Check sheet for the drawn part. Datum: minimum x, y, z corner. Units: mm. Round coordinates to 2 decimals unless told otherwise and drop trailing zeros. Loops run counter-clockwise (first coordinate to the right, second up) from the corner with the lowest first, then second, coordinate; pieces in that order, holes last. Notation, with made-up numbers: (74.5, 70.5) -> (127.5, 70.5) arc R24 cw to (127.5, 85.5) -> close; hole circle Ø5 at (-7, 45). An arc over 180 degrees is marked (long way). Return JSON: item names as keys, results as strings.
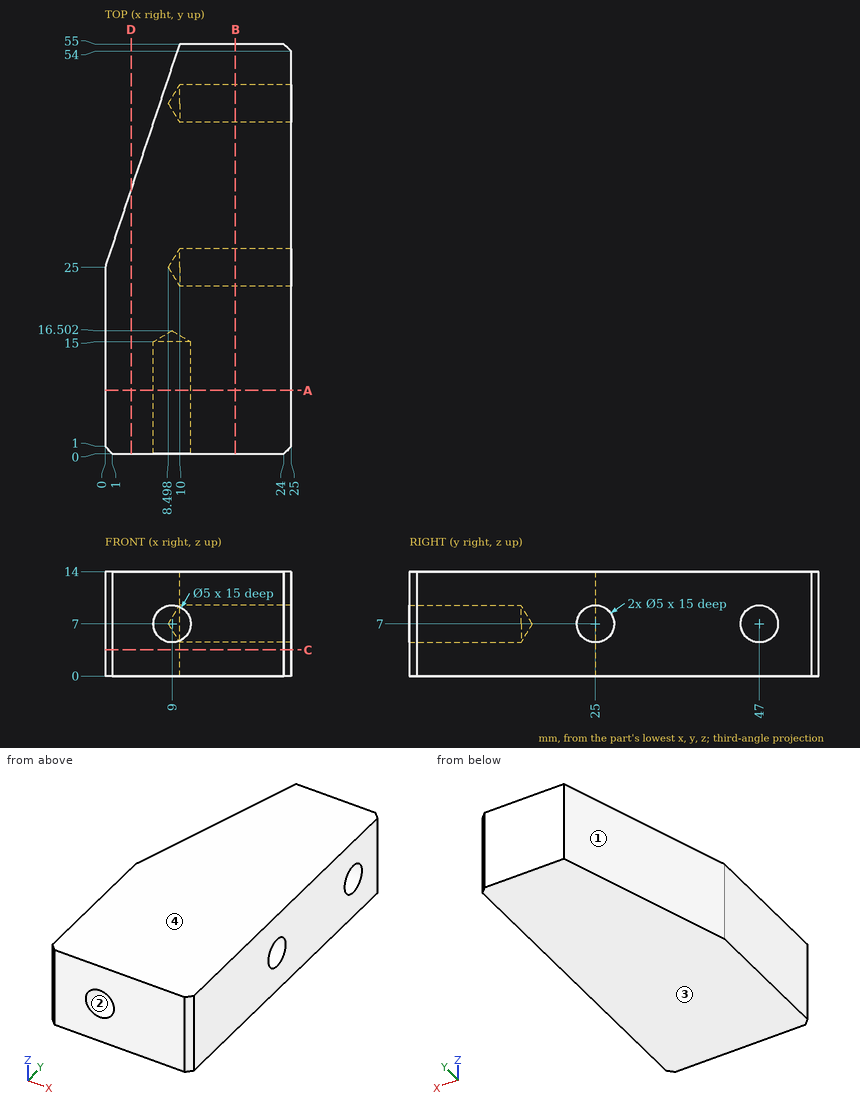
Q1. Section check B-B (x = 17.5). Record the boundary of the cut face in (y, z).
Results list:
{"outline": "(0, 0) -> (55, 0) -> (55, 14) -> (0, 14) -> close; hole circle Ø5 at (25, 7); hole circle Ø5 at (47, 7)"}
Q2. Section check C-C (z = 3.5). Record the boundary of the cut face in (x, y).
Results list:
{"outline": "(0, 1) -> (1, 0) -> (24, 0) -> (25, 1) -> (25, 54) -> (24, 55) -> (10, 55) -> (0, 25) -> close"}
Q3. Draft check along Z on the marked faces 1, 2, 3 and 4. Enter one of: released by +Z, released by -Z, zero draft, split by the parting line, or undercut.
Results list:
{"face 1": "zero draft", "face 2": "undercut", "face 3": "released by -Z", "face 4": "released by +Z"}
Q4. Section check A-A (y = 8.5). Record the boundary of the cut face in (x, z), then the cut area to 3 significant figures.
Results list:
{"outline": "(0, 0) -> (25, 0) -> (25, 14) -> (0, 14) -> close; hole circle Ø5 at (9, 7)", "area": "330 mm^2"}
Q5. Section check D-D (x = 3.5). Record the boundary of the cut face in (y, z), then the cut area to 3 significant figures.
Results list:
{"outline": "(0, 0) -> (35.5, 0) -> (35.5, 14) -> (0, 14) -> close", "area": "497 mm^2"}
Q6. Go/stop test with flat-tipped pins: pin 1 (4 mm diameter, centred on x = 9, z = 7, fed in from -Y); pin 2 (4.5 mm diameter, centred on y = 25, z = 7, fed in from -X); pin 3 (1 mm diameter, centred on y = 34.5, z = 8.5, fed in from -X); pin 4 (4 mm diameter, centred on y = 47, z = 7, fed in from -X). Record where each tip stops, or that it passes through.
Results list:
{"pin 1": "y = 15.3", "pin 2": "x = 0", "pin 3": "x = 3", "pin 4": "x = 6.67"}
Q7. Material ranges on line 1 (Y direction, x = 14.5, z = 7); line 2 (Z direction, x = 18.75, y = 25); line 3 (Y direction, x = 12, z = 9), recorded low to high.
Results list:
{"line 1": "0 to 22.5, 27.5 to 44.5, 49.5 to 55", "line 2": "0 to 4.5, 9.5 to 14", "line 3": "0 to 23.5, 26.5 to 45.5, 48.5 to 55"}
